Verification items for this drawing (mm, ordinates from the low corner). A direction names the side the tool comes from. Round coordinates to 2 decimals unless told otherwise and drop trailing zeros. Order: outer loops, then holes, each group sorted by start corner. A loop starts at its lowest first (then second) coordinate and runs counter-clockwise, first axis right, second up. Notation, with made-up numbers: M 43,14 L 93,14 A16 cw 93,40 Z; hole C 46.5,-6 d6. An arc over 180 degrees is marked long. One line per item, written item: value. Start each with the question number.
(1) Depth check by flat-ended pin: pin 1 Ø3 at (y, z) = (5, 24.5) entering from +X; pin 2 Ø1.5 at (y, z) = (20, 13) entering from +X; pin 3 Ø2 at (y, z) = (24.5, 5) entering from +X; pin 4 Ø2.5 at (y, z) = (24.5, 44) entering from +X. Enter the tip coordinate at first touch or a pass-through.
(2) Access from +Z, -Z, +X, -X, +Y, -Y to the whole of each face (thin tool, end or side, straight path). Record for the marked faces 4, 5 and 6.
(3) Cross-section at C-C, the plane z = 20.5. Enter the section's corners in (x, y).
(4) Thickness scan on L1, parallel to Z at x = 42, y = 36; L2, parallel to Y at x = 30, z = 24; L3, parallel to X at y = 35.5, z = 43. Record the ranges inside material, lowest first.
(5) Cross-section at B-B, the plane x = 18. Enter the section's corners in (y, z).
(6) Cross-section at D-D, the plane y = 41.5. Enter the section's corners in (x, z), and give its area (3 significant figures).
(7) Release check for a two-part mould opening along Y. For the marked faces 1, 2 and 3 record: released by +Y, released by -Y, zero draft, split by the parting line, or undercut.
(8) Cross-section at A-A, the plane y = 35. Enter the section's corners in (x, z).
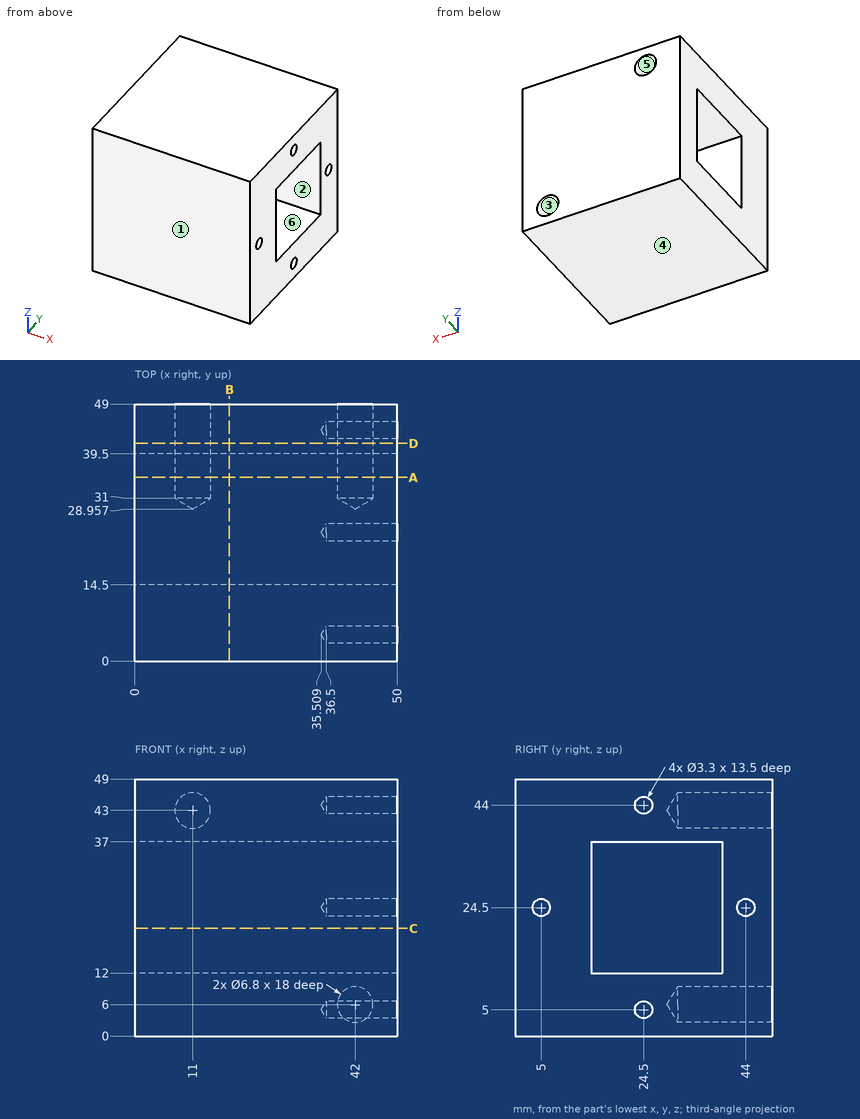
Values found:
1. pin 1: x = 36.41
1. pin 2: through
1. pin 3: x = 36.11
1. pin 4: x = 36.26
2. face 4: -Z, +X, -X, +Y, -Y
2. face 5: +Y
2. face 6: +X, -X
3. outline: M 0,0 L 50,0 L 50,14.5 L 0,14.5 Z; M 0,39.5 L 50,39.5 L 50,49 L 0,49 Z
4. L1: 0 to 2.6, 9.4 to 12, 37 to 49
4. L2: 0 to 14.5, 39.5 to 49
4. L3: 0 to 7.6, 14.4 to 50
5. outline: M 0,0 L 49,0 L 49,49 L 0,49 Z; hole M 14.5,12 L 39.5,12 L 39.5,37 L 14.5,37 Z
6. outline: M 0,0 L 50,0 L 50,49 L 0,49 Z; hole C 11,43 d6.8; hole C 42,6 d6.8
6. area: 2,380 mm^2
7. face 1: released by -Y
7. face 2: undercut
7. face 3: zero draft
8. outline: M 0,0 L 50,0 L 50,12 L 0,12 Z; M 0,37 L 50,37 L 50,49 L 0,49 Z; hole C 11,43 d6.8; hole C 42,6 d6.8
